Read the model definition and answer for the solid it produces. Units are mm, in the model's axes. A direction names the side the tool comes from. Give positions to 0.01 mm unless a question says otherwise; leave off trailing zeros. Order: outer loops, then holes, each group sorted by start corner. A loop starts at its lowest first (then second) coordinate and runs counter-clockwise, first axis right, second up. Notation, with made-up numbers: (80.5, 60.25) - (88.5, 60.25) arc R25 cw to (88.5, 80.25) - close; hole circle Ø1 at (-2, 59). An arc over 180 degrees is marked (long way). Use a Markdown table: item, result. Add a question column.
1. A cutting plane is placed at A-A on z = -51. Determine the outline of the cut face in (x, y).
2. For a pull along X with two mould halves and no side action, classify faces 1 (the flat face through (217, 110, -116)), 2 (the cylindrical face through (-275.383, 194.79, -25.858)), 3 (the flat face through (200, 99, -18)) as released by +X, released by -X, zero draft, split by the parting line, or undercut.
3. A cutting plane is placed at B-B on z = 88. Determine the outline of the cut face in (x, y), and give its area (3 significant figures).
4. Flat-ended cylindrical pins translate along their axes: P1, Ø3, axis at y = 204, z = -58, coming from the +X side; P2, Ø15, axis at x = -219, y = 5.5, coming from the -Z side; P3, Ø1, axis at x = 65, z = -51, coming from the -Y side. Find the tip coordinate at first contact, or state that the pin passes through.
5. Which of the six approach directions +Z, -Z, +X, -X, +Y, -Y give full straight-line access (tool end or side, diameter ignored) to faces 4 (the flat face through (217, 90, -116)), 5 (the flat face through (-276, 20, -39)), 6 (the flat face through (220, 100, 110))?
6. A cutting plane is placed at D-D on y = 169. Determine the outline of the cut face in (x, z).
7. A cutting plane is placed at C-C on x = -286. Determine the outline of the cut face in (y, z), and give its area (3 significant figures).
8. Consider L1, parallel to X at y = 88, z = 88; L2, parallel to X at y = 8, z = -20; L3, parallel to Y at x = -291, z = -89.5. Determine where each line is inside the solid, lowest interval first.
```python
from build123d import *

# Parameters (mm, degrees)
SKETCH1_W                = 400
SKETCH1_H                = 300
BOSS_EXTRUDE1_DEPTH      = 200
BOSS_EXTRUDE2_DEPTH      = 29
BOSS_EXTRUDE2_DEPTH_BACK = 29
SKETCH2_R                = 15
CUT_EXTRUDE1_DEPTH       = 363.138095207
BOSS_EXTRUDE3_START      = -20
SKETCH4_R                = 45
BOSS_EXTRUDE3_DEPTH      = 30
BOSS_EXTRUDE4_DEPTH      = 10
BOSS_EXTRUDE4_DEPTH_BACK = 10
SKETCH5_R                = 13


with BuildPart() as part:
    # Sketch1 → Boss-Extrude1 (new body)
    with BuildSketch(Plane(origin=(0, 0, 0), x_dir=(1, 0, 0), z_dir=(0, 1, 0))):
        Rectangle(SKETCH1_W, SKETCH1_H)
    extrude(amount=BOSS_EXTRUDE1_DEPTH)

    # Sketch2 → Boss-Extrude2 (add, two sides: drawn at the far end of the back side and taken through both)
    with BuildSketch(Plane(origin=(0, 100, 0), x_dir=(1, 0, 0), z_dir=(0, 1, 0)).offset(-BOSS_EXTRUDE2_DEPTH_BACK)):
        with BuildLine():
            Line((187.36144438, -66), (240, -66))
            ThreePointArc((240, -66), (262, -88), (240, -110))
            Line((240, -110), (187.36144438, -110))
            Line((187.36144438, -110), (187.36144438, -66))
        make_face()
        with Locations(Location((240, -88, 0), (0, 0, 270))):
            Circle(SKETCH2_R, mode=Mode.SUBTRACT)
    extrude(amount=BOSS_EXTRUDE2_DEPTH + BOSS_EXTRUDE2_DEPTH_BACK)

    # Sketch3 → Cut-Extrude1 (cut, through all)
    with BuildSketch(Plane(origin=(0, 200, 0), x_dir=(1, 0, 0), z_dir=(0, 1, 0))):
        Polygon((200, -110), (20.728700198, -150), (200, -150), align=None)
    extrude(amount=-CUT_EXTRUDE1_DEPTH, mode=Mode.SUBTRACT)

    # Sketch4 → Boss-Extrude3 (add)
    with BuildSketch(Plane(origin=(0, 200, 0), x_dir=(1, 0, 0), z_dir=(0, 1, 0)).offset(BOSS_EXTRUDE3_START)):
        with BuildLine():
            Line((-94.278565111, -60), (-320, -60))
            ThreePointArc((-320, -60), (-400, 20), (-320, 100))
            Line((-320, 100), (-94.278565111, 100))
            Line((-94.278565111, 100), (-94.278565111, -60))
        make_face()
        with Locations(Location((-320, 20, 0), (0, 0, 270))):
            Circle(SKETCH4_R, mode=Mode.SUBTRACT)
    boss_extrude3 = extrude(amount=BOSS_EXTRUDE3_DEPTH)

    # Mirror1: Boss-Extrude3 across plane
    add(boss_extrude3.mirror(Plane.ZX.offset(100)))

    # Sketch5 → Boss-Extrude4 (add, two sides: drawn at the far end of the back side and taken through both)
    with BuildSketch(Plane(origin=(0, 100, 0), x_dir=(1, 0, 0), z_dir=(0, 1, 0)).offset(-BOSS_EXTRUDE4_DEPTH_BACK)):
        with BuildLine():
            Line((184.247820943, 140), (235, 140))
            ThreePointArc((235, 140), (259, 116), (235, 92))
            Line((235, 92), (184.247820943, 92))
            Line((184.247820943, 92), (184.247820943, 140))
        make_face()
        with Locations(Location((235, 116, 0), (0, 0, 270))):
            Circle(SKETCH5_R, mode=Mode.SUBTRACT)
    extrude(amount=BOSS_EXTRUDE4_DEPTH + BOSS_EXTRUDE4_DEPTH_BACK)


solid = part.part
```
Output values:
| question | item | result |
|---|---|---|
| 1 | outline | (-393.75, -10) - (-352.62, -10) - (-352.62, 20) - (-393.75, 20) - close; (-393.75, 180) - (-352.62, 180) - (-352.62, 210) - (-393.75, 210) - close; (-287.38, -10) - (-94.28, -10) - (-94.28, 0) - (200, 0) - (200, 200) - (-94.28, 200) - (-94.28, 210) - (-287.38, 210) - (-287.38, 180) - (-200, 180) - (-200, 20) - (-287.38, 20) - close |
| 2 | face 1 | zero draft |
| 2 | face 2 | undercut |
| 2 | face 3 | released by +X |
| 3 | outline | (-200, 0) - (200, 0) - (200, 71) - (225, 71) - (225, 129) - (200, 129) - (200, 200) - (-200, 200) - close; (255, 71) - (262, 71) - (262, 129) - (255, 129) - close |
| 3 | area | 81,900 mm² |
| 4 | P1 | x = -94.28 |
| 4 | P2 | z = -100 |
| 4 | P3 | y = 0 |
| 5 | face 4 | -Z, +X, -Y |
| 5 | face 5 | +Z, -Z, -X |
| 5 | face 6 | +Z, +X, +Y, -Y |
| 6 | outline | (-200, -150) - (200, -150) - (200, 110) - (20.73, 150) - (-200, 150) - close |
| 7 | outline | (-10, -100) - (20, -100) - (20, -49.48) - (-10, -49.48) - close; (-10, 9.48) - (20, 9.48) - (20, 60) - (-10, 60) - close; (180, -100) - (210, -100) - (210, -49.48) - (180, -49.48) - close; (180, 9.48) - (210, 9.48) - (210, 60) - (180, 60) - close |
| 7 | area | 6,060 mm² |
| 8 | L1 | -200 to 225, 255 to 262 |
| 8 | L2 | -400 to -365, -275 to 200 |
| 8 | L3 | -10 to 20, 180 to 210 |
